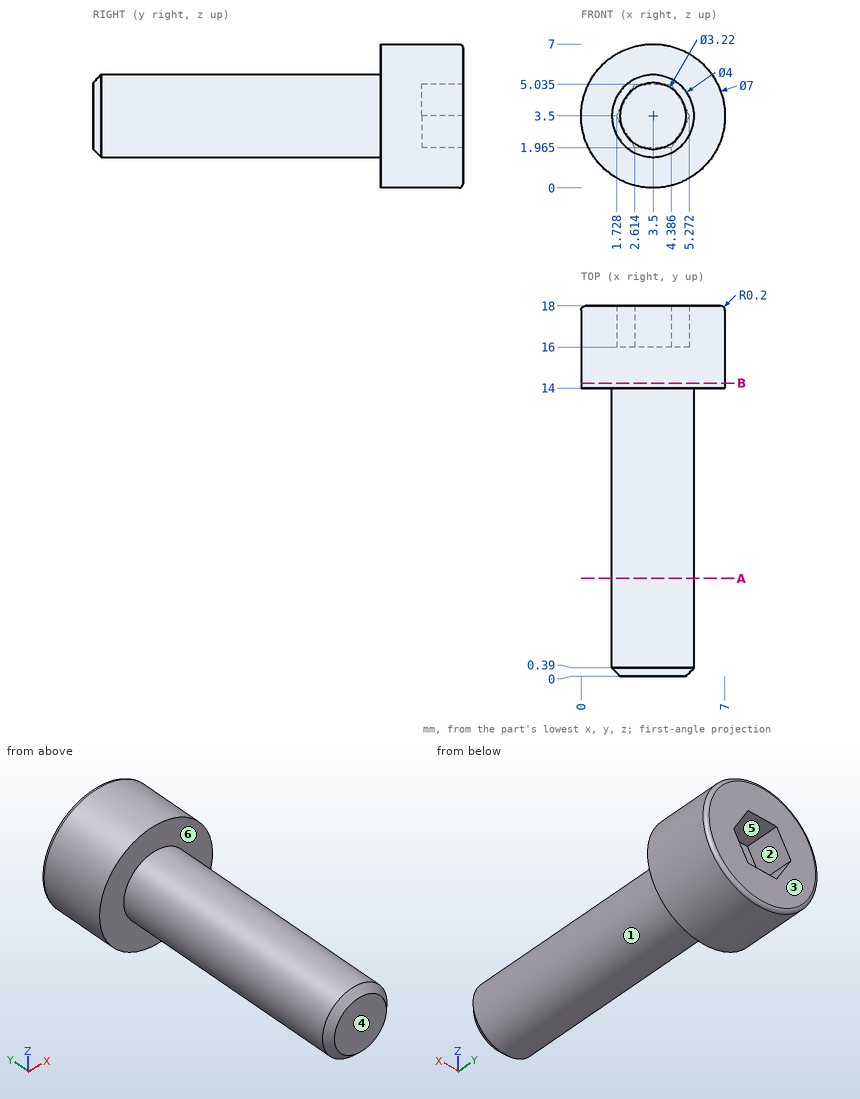
Source: three-view drawing plus pictorial views. Frame: mm from the lowest corner of the part. A direction names the side the tool comes from. Coordinates: 2 decimals unless noted, no trailing zeros. Write each loop counter-clockwise with the first axis right and the second up, starting at its lowest first coordinate (ties: lowest second). Pieces come first, ordered by that corner, then holes. Notation, with made-up numbers: (16, 40) - (27, 40) arc R15 cw to (27, 69) - close; hole circle Ø3 at (-3.5, -30). An arc over 180 degrees is marked (long way). Answer as a JSON object with one key per item and string values.
Q1. Set-up query: the marked faces 4, 5 and 6. Return all of +Z, -Z, +X, -X, +Y, -Y with unobstructed straight access to the full face (end or side cutting, diameter ignored); none if empty.
Ans:
{"face 4": "+Z, -Z, +X, -X, -Y", "face 5": "+Y", "face 6": "-Y"}
Q2. Material intervals for line 1 (Y direction, x = 1.25, z = 4); line 2 (Y direction, x = 2.75, z = 2.75); line 3 (Z direction, x = 5, y = 17) (1 decimal), sorted ascending. Write a range as [from, to].
Ans:
{"line 1": "y = [14, 18]", "line 2": "y = [0, 16]", "line 3": "z = [0.3, 3], [4, 6.7]"}
Q3. Section query B-B, the plane y = 14.25. Output: boundary loops of the cut face in (x, z), plus the area to 3 significant figures.
Ans:
{"outline": "circle Ø7 at (3.5, 3.5)", "area": "38.5 mm2"}
Q4. First-contact query: pin 1 Ø4 at (x, y) = (4, 4.5) entering from +Z; pin 2 Ø1.5 at (x, y) = (5, 10.5) entering from -Z (1 decimal); pin 3 Ø4 at (y, z) = (8, 1) entering from -X. Flat tips, straight axial feed; report the tip coordinate or a pass-through.
Ans:
{"pin 1": "stops at z = 5.5", "pin 2": "stops at z = 1.6", "pin 3": "stops at x = 1.56"}
Q5. Section query A-A, the plane y = 4.75. Output: boundary loops of the cut face in (x, z).
Ans:
{"outline": "circle Ø4 at (3.5, 3.5)"}
Q6. Draft query along Z for the marked faces 1, 2 and 3. Return one class per face: released by +Z, released by -Z, zero draft, split by the parting line, or undercut.
Ans:
{"face 1": "split by the parting line", "face 2": "undercut", "face 3": "zero draft"}
